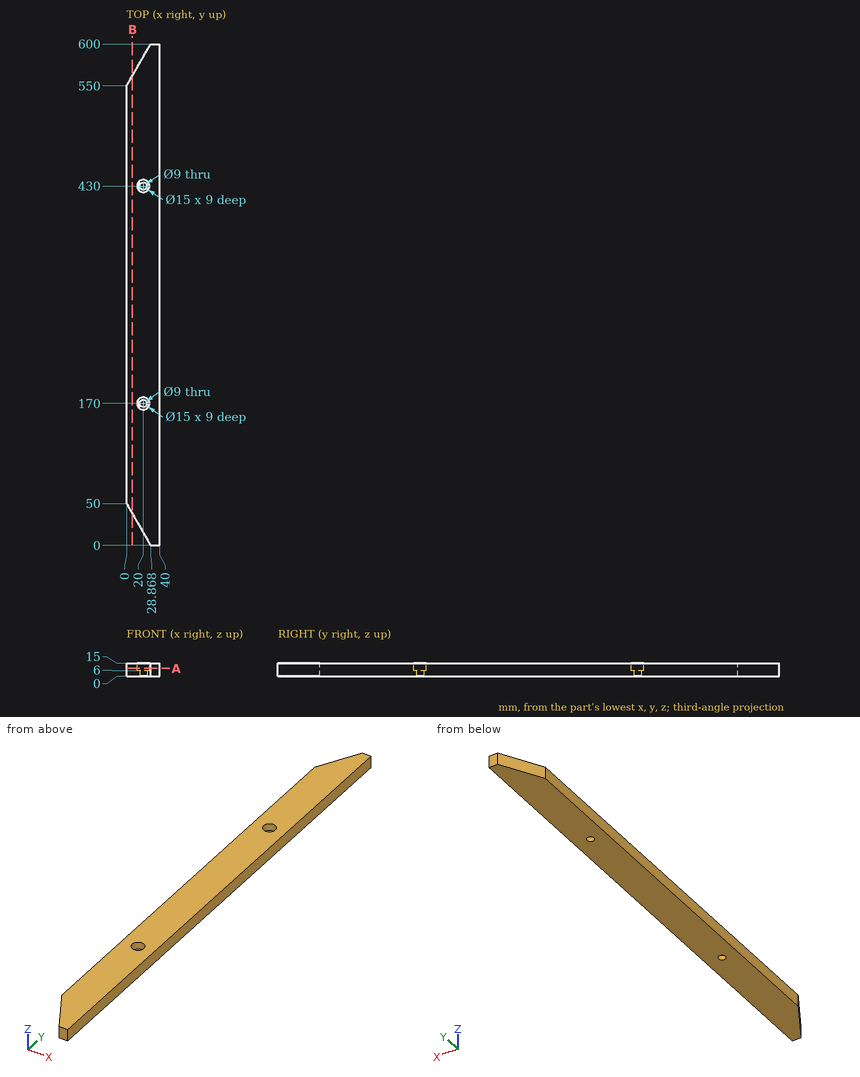
Here's the drawing with two shaded views (mm, measured from the low corner). I have some questions. Give positions to 0.01 mm unless a question says otherwise; leave off trailing zeros. Loops run counter-clockwise (first coordinate to the right, second up) from the corner with the lowest first, then second, coordinate; pieces in that order, holes last. Notation, with made-up numbers: M -35,82.5 L -27,82.5 A19 cw -27,100.5 Z; hole C -1,62 d6. An arc over 180 degrees is marked long. One line per item, written item: value. Start each with the question number.
1) If we section it at B-B, the plane x = 7: Write out the boundary of the cut face in (y, z) (1 decimal), and give its area (3 significant figures).
2) If I drill on line 1 (X direction, y = 170, z = 13); line 2 (Y direction, x = 23, z = 6.25) (1 decimal); line 3 (Y direction, x = 17, z = 13.75) (1 decimal), over which ranges is the centre line in solid material (lowest first)? Write a range as [from, to].
3) I'm going to push flat-ended pins straight in: pin 1 (3 mm diameter, centred on x = 12.5, z = 9, fed in from +Y); pin 2 (1 mm diameter, centred on x = 26.5, z = 10, fed in from -Y) (1 decimal); pin 3 (7.5 mm diameter, centred on x = 19, y = 172.5, fed in from +Z). Where does each tip first touch, or does it pass through?
4) If we section it at A-A, the plane z = 9: Write out the boundary of the cut face in (x, y).
Completed:
1. outline: M 37.9,0 L 562.1,0 L 562.1,15 L 37.9,15 Z
1. area: 7,860 mm^2
2. line 1: x = [0, 12.5], [27.5, 40]
2. line 2: y = [10.2, 163.1], [176.9, 423.1], [436.9, 589.8]
2. line 3: y = [20.6, 163.1], [176.9, 423.1], [436.9, 579.4]
3. pin 1: stops at y = 574.25
3. pin 2: stops at y = 3.2
3. pin 3: stops at z = 6
4. outline: M 0,50 L 28.87,0 L 40,0 L 40,600 L 28.87,600 L 0,550 Z; hole C 20,170 d15; hole C 20,430 d15
